```python
from build123d import *

# Parameters (mm, degrees)
SKETCH_1_W      = 30
SKETCH_1_H      = 50
SKETCH_1_W_2    = 24
SKETCH_1_H_2    = 44
EXTRUDE_1_DEPTH = 100


with BuildPart() as part:
    # 草图1 → 凸台-拉伸1 (new, symmetric)
    with BuildSketch(Plane.XY):
        Rectangle(SKETCH_1_W, SKETCH_1_H)
        Rectangle(SKETCH_1_W_2, SKETCH_1_H_2, mode=Mode.SUBTRACT)
    extrude(amount=EXTRUDE_1_DEPTH, both=True)


solid = part.part
```
The listing builds one solid part. Answer for the finished solid, in the listing's coordinates (mm). A direction names the side the tool comes from. Round coordinates to 2 decimals unless told otherwise and drop trailing zeros. Loops run counter-clockwise (first coordinate to the right, second up) from the corner with the lowest first, then second, coordinate; pieces in that order, holes last.
Q1. Section C-C, the plane x = 5 is taken. Determine the outline of the cut face in (y, z).
Q2. For a pull along Y with two mould halves and no side action, classify faces 3 (the face through (-15, 0, 1)), 4 (the face through (-12, 0, 1)), 5 (the face through (0, 25, 1)) as released by +Y, released by -Y, zero draft, split by the parting line, or undercut.
Q3. Which of the six approach directions +Z, -Z, +X, -X, +Y, -Y give full straight-line access (tool end or side, diameter ignored) to faces 1 (the face through (0, 22, 1)), 2 (the face through (-12.3, -1.7, 100))?
Q4. Section B-B, the plane z = -45.5 is taken. Determine the outline of the cut face in (x, y), then the cut area to 3 significant figures.
Q5. Section A-A, the plane y = -1 is taken. Determine the outline of the cut face in (x, z).
Q6. Find the intervals of material crossed by line 1 (X direction, y = 20, z = -72); line 2 (Y direction, x = 11.5, z = 24.5), in increasing order.
Completed:
1. outline: (-25, -100) - (-22, -100) - (-22, 100) - (-25, 100) - close; (22, -100) - (25, -100) - (25, 100) - (22, 100) - close
2. face 3: zero draft
2. face 4: undercut
2. face 5: released by +Y
3. face 1: +Z, -Z
3. face 2: +Z, +X, -X, +Y, -Y
4. outline: (-15, -25) - (15, -25) - (15, 25) - (-15, 25) - close; hole (-12, -22) - (12, -22) - (12, 22) - (-12, 22) - close
4. area: 444 mm2
5. outline: (-15, -100) - (-12, -100) - (-12, 100) - (-15, 100) - close; (12, -100) - (15, -100) - (15, 100) - (12, 100) - close
6. line 1: x = -15 to -12, 12 to 15
6. line 2: y = -25 to -22, 22 to 25
